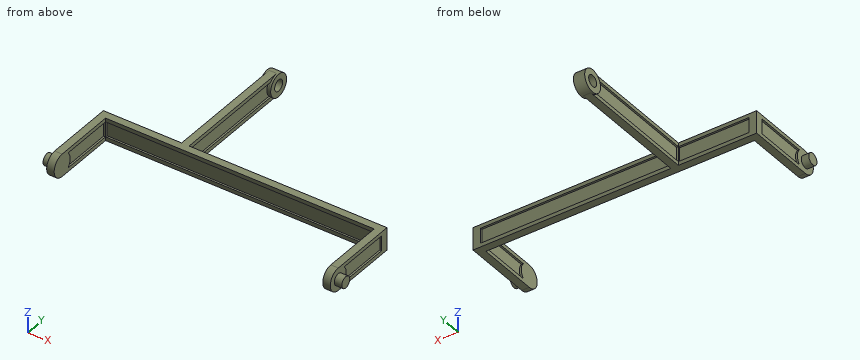
```python
from build123d import *

# Parameters (mm, degrees)
SKETCH_2_R           = 30
SKETCH_2_R_2         = 15
EXTRUDE_1_DEPTH      = 15
EXTRUDE_2_DEPTH      = 10
CUT_EXTRUDE_1_DEPTH  = 5
CUT_EXTRUDE_START    = -5
CUT_EXTRUDE_2_DEPTH  = 5
EXTRUDE_3_DEPTH      = 536
EXTRUDE_3_DEPTH_BACK = 218
SKETCH_6_W           = 60
SKETCH_6_H           = 20
SKETCH_8_W           = 188
SKETCH_8_H           = 40
SKETCH_8_W_2         = 506
CUT_EXTRUDE_3_DEPTH  = 5
SKETCH_9_W           = 714
SKETCH_9_H           = 40
CUT_EXTRUDE_4_DEPTH  = 5
EXTRUDE_4_DEPTH      = 20
EXTRUDE_START        = -20
EXTRUDE_5_DEPTH      = 20
CUT_EXTRUDE_5_DEPTH  = 5
CUT_EXTRUDE_6_DEPTH  = 5
CUT_EXTRUDE_7_DEPTH  = 5
CUT_EXTRUDE_8_DEPTH  = 5
SKETCH_17_R          = 15
EXTRUDE_6_DEPTH      = 20
SKETCH_18_R          = 15.5
EXTRUDE_7_DEPTH      = 20


with BuildPart() as part:
    # 草图2 → 凸台-拉伸1 (new, symmetric)
    with BuildSketch(Plane(origin=(0, 0, 0), x_dir=(0, 0, -1), z_dir=(1, 0, 0))):
        with Locations((0, 34.284448819)):
            Circle(SKETCH_2_R)
        with Locations((0, 34.284448819)):
            Circle(SKETCH_2_R_2, mode=Mode.SUBTRACT)
    extrude(amount=EXTRUDE_1_DEPTH, both=True)

    # 草图3 → 凸台-拉伸2 (add, symmetric)
    with BuildSketch(Plane(origin=(0, 0, 0), x_dir=(0, 0, -1), z_dir=(1, 0, 0))):
        with BuildLine():
            Line((-30, 34.284448819), (-30, -315.715551181))
            Line((-30, -315.715551181), (30, -315.715551181))
            Line((30, -315.715551181), (30, 34.284448819))
            ThreePointArc((30, 34.284448819), (0, 4.284448819), (-30, 34.284448819))
        make_face()
    extrude(amount=EXTRUDE_2_DEPTH, both=True)

    # 草图4 → 切除-拉伸1 (cut)
    with BuildSketch(Plane(origin=(10, 0, 0), x_dir=(0, 0, -1), z_dir=(1, 0, 0))):
        with BuildLine():
            Line((-20, -315.715551181), (-20, 11.923769044))
            ThreePointArc((-20, 11.923769044), (0, 4.284448819), (20, 11.923769044))
            Line((20, 11.923769044), (20, -315.715551181))
            Line((20, -315.715551181), (-20, -315.715551181))
        make_face()
    extrude(amount=-CUT_EXTRUDE_1_DEPTH, mode=Mode.SUBTRACT)

    # 草图5 → 切除-拉伸2 (cut)
    with BuildSketch(Plane.ZY.offset(10).offset(CUT_EXTRUDE_START)):
        with BuildLine():
            Line((-20, 11.923769044), (-20, -315.715551181))
            Line((-20, -315.715551181), (20, -315.715551181))
            Line((20, -315.715551181), (20, 11.923769044))
            ThreePointArc((20, 11.923769044), (0, 4.284448819), (-20, 11.923769044))
        make_face()
    extrude(amount=CUT_EXTRUDE_2_DEPTH, mode=Mode.SUBTRACT)

    # 草图6 → 凸台-拉伸3 (add, two sides: drawn at the far end of the back side and taken through both)
    with BuildSketch(Plane(origin=(0, 0, 0), x_dir=(0, 0, -1), z_dir=(1, 0, 0)).offset(-EXTRUDE_3_DEPTH_BACK)):
        with Locations((0, -305.715551181)):
            Rectangle(SKETCH_6_W, SKETCH_6_H)
    extrude(amount=EXTRUDE_3_DEPTH + EXTRUDE_3_DEPTH_BACK)

    # 草图8 → 切除-拉伸3 (cut)
    with BuildSketch(Plane(origin=(0, -295.715551181, 0), x_dir=(1, 0, 0), z_dir=(0, 1, 0))):
        with Locations((-104, 0)):
            Rectangle(SKETCH_8_W, SKETCH_8_H)
        with Locations((263, 0)):
            Rectangle(SKETCH_8_W_2, SKETCH_8_H)
    extrude(amount=-CUT_EXTRUDE_3_DEPTH, mode=Mode.SUBTRACT)

    # 草图9 → 切除-拉伸4 (cut)
    with BuildSketch(Plane.XZ.offset(315.715551181)):
        with Locations((159, 0)):
            Rectangle(SKETCH_9_W, SKETCH_9_H)
    extrude(amount=-CUT_EXTRUDE_4_DEPTH, mode=Mode.SUBTRACT)

    # 草图11 → 凸台-拉伸4 (add)
    with BuildSketch(Plane(origin=(536, 0, 0), x_dir=(0, 0, -1), z_dir=(1, 0, 0))):
        with BuildLine():
            Line((30, -479.215551181), (30, -315.715551181))
            Line((30, -315.715551181), (-30, -315.715551181))
            Line((-30, -315.715551181), (-30, -479.215551181))
            ThreePointArc((-30, -479.215551181), (0, -509.215551181), (30, -479.215551181))
        make_face()
    extrude(amount=-EXTRUDE_4_DEPTH)

    # 草图12 → 凸台-拉伸5 (add)
    with BuildSketch(Plane.ZY.offset(218).offset(EXTRUDE_START)):
        with BuildLine():
            Line((-30, -315.715551181), (30, -315.715551181))
            Line((30, -315.715551181), (30, -479.215551181))
            ThreePointArc((30, -479.215551181), (0, -509.215551181), (-30, -479.215551181))
            Line((-30, -479.215551181), (-30, -315.715551181))
        make_face()
    extrude(amount=EXTRUDE_5_DEPTH)

    # 草图13 → 切除-拉伸5 (cut)
    with BuildSketch(Plane.ZY.offset(218).offset(CUT_EXTRUDE_START)):
        with BuildLine():
            Line((-20, -315.715551181), (20, -315.715551181))
            Line((20, -315.715551181), (20, -456.854871406))
            ThreePointArc((20, -456.854871406), (0, -449.215551181), (-20, -456.854871406))
            Line((-20, -456.854871406), (-20, -315.715551181))
        make_face()
    extrude(amount=CUT_EXTRUDE_5_DEPTH, mode=Mode.SUBTRACT)

    # 草图14 → 切除-拉伸6 (cut)
    with BuildSketch(Plane(origin=(-198, 0, 0), x_dir=(0, 0, -1), z_dir=(1, 0, 0))):
        with BuildLine():
            Line((-20, -456.854871406), (-20, -315.715551181))
            Line((-20, -315.715551181), (20, -315.715551181))
            Line((20, -315.715551181), (20, -456.854871406))
            ThreePointArc((20, -456.854871406), (0, -449.215551181), (-20, -456.854871406))
        make_face()
    extrude(amount=-CUT_EXTRUDE_6_DEPTH, mode=Mode.SUBTRACT)

    # 草图15 → 切除-拉伸7 (cut)
    with BuildSketch(Plane(origin=(536, 0, 0), x_dir=(0, 0, -1), z_dir=(1, 0, 0))):
        with BuildLine():
            Line((-20, -456.854871406), (-20, -315.715551181))
            Line((-20, -315.715551181), (20, -315.715551181))
            Line((20, -315.715551181), (20, -456.854871406))
            ThreePointArc((20, -456.854871406), (0, -449.215551181), (-20, -456.854871406))
        make_face()
    extrude(amount=-CUT_EXTRUDE_7_DEPTH, mode=Mode.SUBTRACT)

    # 草图16 → 切除-拉伸8 (cut)
    with BuildSketch(Plane.ZY.offset(-516).offset(CUT_EXTRUDE_START)):
        with BuildLine():
            Line((-20, -456.854871406), (-20, -315.715551181))
            Line((-20, -315.715551181), (20, -315.715551181))
            Line((20, -315.715551181), (20, -456.854871406))
            ThreePointArc((20, -456.854871406), (0, -449.215551181), (-20, -456.854871406))
        make_face()
    extrude(amount=CUT_EXTRUDE_8_DEPTH, mode=Mode.SUBTRACT)

    # 草图17 → 凸台-拉伸6 (add)
    with BuildSketch(Plane(origin=(536, 0, 0), x_dir=(0, 0, -1), z_dir=(1, 0, 0))):
        with Locations(Location((0, -479.215551181, 0), (0, 0, 180))):
            Circle(SKETCH_17_R)
    extrude(amount=EXTRUDE_6_DEPTH)

    # 草图18 → 凸台-拉伸7 (add)
    with BuildSketch(Plane.ZY.offset(218)):
        with Locations((0, -479.215551181)):
            Circle(SKETCH_18_R)
    extrude(amount=EXTRUDE_7_DEPTH)


solid = part.part
```
Could you check a few things on this model? Use its own coordinates, in mm. Coordinates: 2 decimals unless noted, no trailing zeros. Loops run counter-clockwise (first coordinate to the right, second up) from the corner with the lowest first, then second, coordinate; pieces in that order, holes last. Notation, with made-up numbers: M 84,-21 L 143,-21 A24 ccw 143,-4 Z; hole C 9.25,48.5 d9. An arc over 180 degrees is marked long. Put each result on its own line as item: value. Start each with the question number.
(1) I need wall thicknesses on line 1 (Y direction, x = 5.5, z = 0); line 2 (X direction, y = -332.5, z = -21); line 3 (Y direction, x = -2, z = 0). Which ranges of each line are inside material? Lowest first, please. Write a range as from..to.
(2) Suppose I cut it at B-B on x = 119.5. Please give me the cut outline in (y, z).
(3) Will these pins go through, and if not, where does the flat tip stop? P1, Ø10, axis at x = 351, z = 7, coming from the -Y side; P2, Ø1, axis at y = -262.5, z = -20.5, coming from the -X side; P3, Ø2.5, axis at x = 533, z = 3, coming from the -Y side; P4, Ø18, axis at y = 34.28, z = 0, coming from the -X side.
(4) Suppose I cut it at A-A on y = -255. Please give me the cut outline in (x, z).
Solutions:
1. line 1: y = -310.72..-295.72, 4.28..19.28, 49.28..64.28
1. line 2: x = -218..-198, 516..536
1. line 3: y = -310.72..19.28, 49.28..64.28
2. outline: M -315.72,-30 L -295.72,-30 L -295.72,-20 L -300.72,-20 L -300.72,20 L -295.72,20 L -295.72,30 L -315.72,30 L -315.72,20 L -310.72,20 L -310.72,-20 L -315.72,-20 Z
3. P1: stops at y = -310.72
3. P2: stops at x = -10
3. P3: stops at y = -509.16
3. P4: passes through
4. outline: M -10,-30 L 10,-30 L 10,-20 L 5,-20 L 5,20 L 10,20 L 10,30 L -10,30 L -10,20 L -5,20 L -5,-20 L -10,-20 Z
